Design review of the part built by this model. Coordinates are the model's own, in mm. Face numbers are marked on the shaded views. A direction names the side the tool comes from. Give positions to 0.01 mm unless a question says otherwise; leave off trailing zeros. Loops run counter-clockwise (first coordinate to the right, second up) from the corner with the lowest first, then second, coordinate; pieces in that order, holes last.
from build123d import *

# Parameters (mm, degrees)
SKETCH1_W                      = 60
SKETCH1_H                      = 90
BOSS_EXTRUDE1_DEPTH            = 10
SKETCH4_R                      = 15
CUT_EXTRUDE3_DEPTH             = 56
M4_TAPPED_HOLE1_D              = 3.3
SKETCH8_W                      = 50
SKETCH8_H                      = 15
CUT_EXTRUDE5_DEPTH             = 56
F_5_5_5_5_DIAMETER_HOLE1_D     = 5.5
F_5_5_5_5_DIAMETER_HOLE1_DEPTH = 12.4
F_5_5_5_5_DIAMETER_HOLE1_TIP   = 1.652366702
FILLET1_R                      = 5
M5_TAPPED_HOLE1_D              = 4.2
M5_TAPPED_HOLE1_DEPTH          = 12.4
M5_TAPPED_HOLE1_TIP            = 1.2618073


with BuildPart() as part:
    # Sketch1 → Boss-Extrude1 (new body)
    with BuildSketch(Plane(origin=(0, 0, 0), x_dir=(1, 0, 0), z_dir=(0, 1, 0))):
        Rectangle(SKETCH1_W, SKETCH1_H)
    extrude(amount=BOSS_EXTRUDE1_DEPTH)

    # Sketch4 → Cut-Extrude3 (cut, through all)
    with BuildSketch(Plane.XZ):
        with Locations(Location((0, -10, 0), (0, 0, 270))):
            Circle(SKETCH4_R)
    extrude(amount=-CUT_EXTRUDE3_DEPTH, mode=Mode.SUBTRACT)

    # M4 Tapped Hole1 (through all)
    with Locations(Plane.XZ):
        with Locations((-24.748737342, 24.747474683), (-24.748737342, -24.75), (24.748737342, -24.75), (24.748737342, 24.747474683)):
            Hole(M4_TAPPED_HOLE1_D / 2)

    # Sketch8 → Cut-Extrude5 (cut, through all)
    with BuildSketch(Plane.XZ):
        with Locations((5, 37.5)):
            Rectangle(SKETCH8_W, SKETCH8_H)
        with Locations((5, -37.5)):
            Rectangle(SKETCH8_W, SKETCH8_H)
    extrude(amount=-CUT_EXTRUDE5_DEPTH, mode=Mode.SUBTRACT)

    # Ø5.5 (5.5) Diameter Hole1
    with Locations(Plane.ZY.offset(30)):
        with Locations((-40, 5), (40, 5)):
            Hole(F_5_5_5_5_DIAMETER_HOLE1_D / 2, depth=F_5_5_5_5_DIAMETER_HOLE1_DEPTH)
            with Locations((0, 0, -(F_5_5_5_5_DIAMETER_HOLE1_DEPTH + F_5_5_5_5_DIAMETER_HOLE1_TIP / 2))):  # 118° drill point
                Cone(0, F_5_5_5_5_DIAMETER_HOLE1_D / 2, F_5_5_5_5_DIAMETER_HOLE1_TIP, mode=Mode.SUBTRACT)

    # Fillet1
    fillet1_edges = [part.edges().sort_by_distance(p)[0] for p in [
        (-20, 5, 30),
        (-20, 5, -30),
    ]]
    fillet(fillet1_edges, radius=FILLET1_R)

    # M5 Tapped Hole1
    with Locations(Plane(origin=(30, 0, 0), x_dir=(0, 0, -1), z_dir=(1, 0, 0))):
        with Locations((-10.000955133, 4.5)):
            Hole(M5_TAPPED_HOLE1_D / 2, depth=M5_TAPPED_HOLE1_DEPTH)
            with Locations((0, 0, -(M5_TAPPED_HOLE1_DEPTH + M5_TAPPED_HOLE1_TIP / 2))):  # 118° drill point
                Cone(0, M5_TAPPED_HOLE1_D / 2, M5_TAPPED_HOLE1_TIP, mode=Mode.SUBTRACT)


solid = part.part
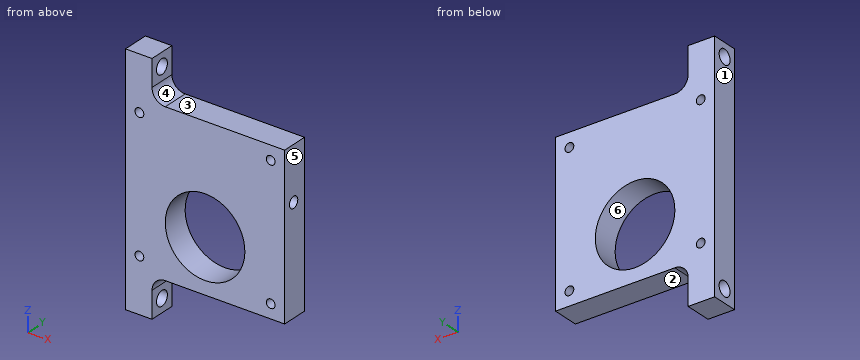
Q1. Insertion check: pin 1 (2 mm diameter, centred on x = 7, y = 6, fed in from -Z); pin 2 (3 mm diameter, centred on x = 12.5, y = 5, fed in from +Z). Each pin has a flat end and moves straight along its axis. Give the tip position at first contact, or say it passes through.
Results:
pin 1: stops at z = -30
pin 2: stops at z = 30
Q2. Take a section at B-B (x = 0). Give the boundary of the cut face in (y, z).
Results:
outline: (0, -30) - (10, -30) - (10, -25) - (0, -25) - close; (0, 5) - (10, 5) - (10, 30) - (0, 30) - close
Q3. Take a section at C-C (y = 1). Give the boundary of the cut face in (x, z), plus the area to 3 significant figures.
Results:
outline: (-30, -45) - (-20, -45) - (-20, -35) arc R5 cw to (-15, -30) - (30, -30) - (30, 30) - (-15, 30) arc R5 cw to (-20, 35) - (-20, 45) - (-30, 45) - close; hole circle Ø3.3 at (-24.75, -24.75); hole circle Ø3.3 at (-24.75, 24.75); hole circle Ø30 at (0, -10); hole circle Ø3.3 at (24.75, -24.75); hole circle Ø3.3 at (24.75, 24.75)
area: 3,170 mm2
Q4. Take a section at A-A (z = -10). Give the boundary of the cut face in (x, y).
Results:
outline: (-30, 0) - (-15, 0) - (-15, 10) - (-30, 10) - close; (15, 0) - (30, 0) - (30, 10) - (15, 10) - close
Q5. Wall thickness on line 1 (Y direction, x = -21, z = 40); line 2 (Z direction, x = -23.5, y = 3.5); line 3 (Z direction, x = -1, y = 3.75): over which ranges is each line inside the solid? List them lowest first.
Results:
line 1: y = 0 to 2.25, 7.75 to 10
line 2: z = -45 to -42.3, -37.7 to -25.83, -23.67 to 23.67, 25.83 to 37.7, 42.3 to 45
line 3: z = -30 to -24.97, 4.97 to 30
Q6. Tool access review of the marked faces 1, 2 and 3: name each direction out of +Z, -Z, +X, -X, +Y, -Y from which nothing blocks a thin tool from reaching the whole face with its end or side.
Results:
face 1: +Z, -Z, -X, +Y, -Y
face 2: -Z, +X, +Y, -Y
face 3: +Z, +X, +Y, -Y
Q7. Draft analysis for pull direction Z (two halves, no side actions). For the marked faces 4, 5 and 6, state which applies: pulls with the +Z half, pulls with the -Z half, needs draft (parallel to the pull), parting line crosses it, or undercut.
Results:
face 4: pulls with the +Z half
face 5: needs draft
face 6: undercut
